Part print with two shaded views. Sizes in mm from the minimum x, y, z corner. A direction names the side the tool comes from. Give positions to 0.01 mm unless a question says otherwise; leave off trailing zeros. Write each loop counter-clockwise with the first axis right and the second up, starting at its lowest first coordinate (ties: lowest second). Pieces come first, ordered by that corner, then holes. Notation, with made-up numbers: M 75,-10 L 96,-10 A10 ccw 96,-5 Z; hole C 35.5,-31.5 d3. An arc over 180 degrees is marked long. One line per item, written item: value. Start each with the question number.
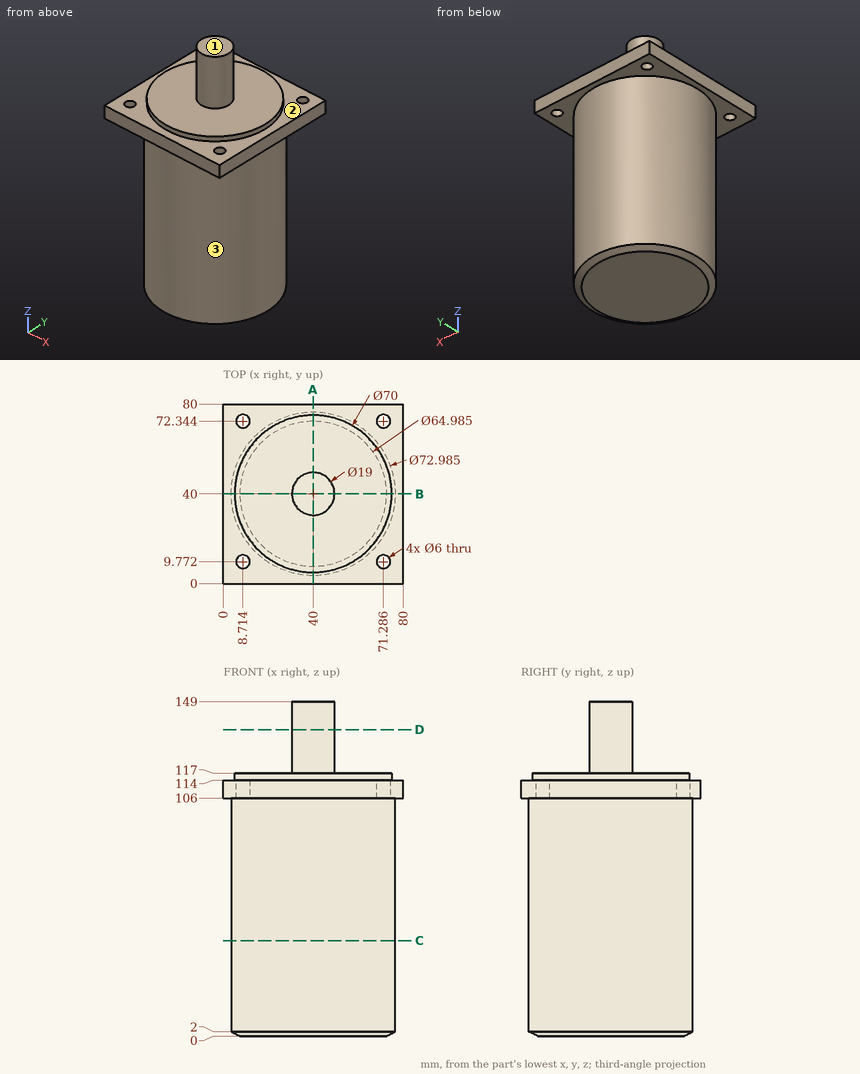
1) Band-saw the part on C-C (z = 42.5). List the corners of the cut face in (x, y) (1 decimal).
2) Band-saw the part on D-D (z = 136.5). List the corners of the cut face in (x, y).
3) Probe line 1 along Z through (x, y) = (60.5, 62.5); line 2 along Z through (x, y) = (67, 68); line 3 along X through (y, z) = (41.5, 100.5). List the from-to ranges inside material, lowest first. Write a range as from..to.
4) Drop flat-ended pins along their axis: P1, Ø2, axis at x = 29, z = 37.5, coming from the -Y side (1 decimal); P2, Ø24, axis at x = 24.5, y = 60, coming from the +Z side; P3, Ø10, axis at x = 48, z = 88, coming from the -Y side. Give the stop position or say it passes through.
5) Tool access for the marked faces 1, 2 and 3: list every direction of +Z, -Z, +X, -X, +Y, -Y with a clear straight run to the whole face (end or side of a thin tool).
6) Band-saw the part on A-A (x = 40). List the corners of the cut face in (y, z).
Model answer:
1. outline: C 40,40 d73
2. outline: C 40,40 d19
3. line 1: z = 0..117
3. line 2: z = 106..114
3. line 3: x = 3.54..76.46
4. P1: stops at y = 4.9
4. P2: stops at z = 117
4. P3: stops at y = 3.63
5. face 1: +Z, +X, -X, +Y, -Y
5. face 2: +Z
5. face 3: -Z
6. outline: M 0,106 L 3.51,106 L 3.51,2 L 7.51,0 L 72.49,0 L 76.49,2 L 76.49,106 L 80,106 L 80,114 L 75,114 L 75,117 L 49.5,117 L 49.5,149 L 30.5,149 L 30.5,117 L 5,117 L 5,114 L 0,114 Z
